Here's the drawing with two shaded views (mm, measured from the low corner). I have some questions. A direction names the side the tool comes from. Coordinates: 2 decimals unless noted, no trailing zeros. Loops run counter-clockwise (first coordinate to the right, second up) from the corner with the lowest first, then second, coordinate; pieces in that order, holes last.
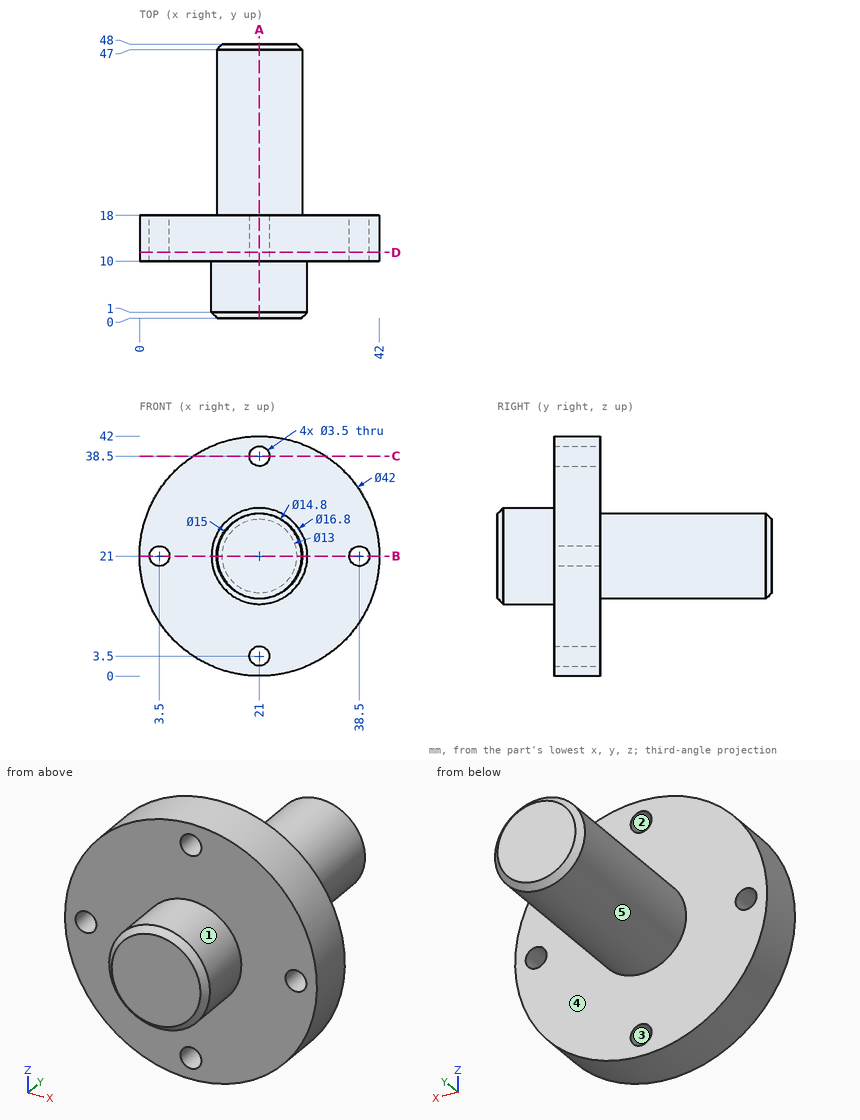
(1) I want a section at B-B on z = 21. Write out the boundary of the cut face in (x, y).
Check values:
outline: (0, 10) - (1.75, 10) - (1.75, 18) - (0, 18) - close; (5.25, 10) - (12.6, 10) - (12.6, 1) - (13.6, 0) - (28.4, 0) - (29.4, 1) - (29.4, 10) - (36.75, 10) - (36.75, 18) - (28.5, 18) - (28.5, 47) - (27.5, 48) - (14.5, 48) - (13.5, 47) - (13.5, 18) - (5.25, 18) - close; (40.25, 10) - (42, 10) - (42, 18) - (40.25, 18) - close
(2) I want a section at C-C on z = 38.5. Write out the boundary of the cut face in (x, y).
Check values:
outline: (9.39, 10) - (19.25, 10) - (19.25, 18) - (9.39, 18) - close; (22.75, 10) - (32.61, 10) - (32.61, 18) - (22.75, 18) - close
(3) I want a section at A-A on x = 21. Write out the boundary of the cut face in (y, z).
Check values:
outline: (0, 13.6) - (1, 12.6) - (10, 12.6) - (10, 5.25) - (18, 5.25) - (18, 13.5) - (47, 13.5) - (48, 14.5) - (48, 27.5) - (47, 28.5) - (18, 28.5) - (18, 36.75) - (10, 36.75) - (10, 29.4) - (1, 29.4) - (0, 28.4) - close; (10, 0) - (18, 0) - (18, 1.75) - (10, 1.75) - close; (10, 40.25) - (18, 40.25) - (18, 42) - (10, 42) - close
(4) If we mould it in two halves opening along X, with no side actions, what happens to the marked faces 3, 4 and 5? For each: released by +X, released by -X, zero draft, split by the parting line, or undercut.
Check values:
face 3: undercut
face 4: zero draft
face 5: split by the parting line
(5) If I drill on probe 1 along X at (y, z) = (12.5, 21); probe 2 along Y at (x, z) = (3.5, 11.5); probe 3 along Z at (x, y) = (39, 14.5), over which ranges is the centre line in solid material (lowest first)?
Check values:
probe 1: x = 0 to 1.75, 5.25 to 36.75, 40.25 to 42
probe 2: y = 10 to 18
probe 3: z = 10.18 to 19.32, 22.68 to 31.82
(6) Which directions (+Z, -Z, +X, -X, +Y, -Y) give clear straight access to the entire face, cutting with the end or side of a thin tool? Please do the marked faces 1 and 2.
Check values:
face 1: -Y
face 2: +Y, -Y
(7) I want a section at D-D on y = 11.5. Write out the boundary of the cut face in (x, z).
Check values:
outline: circle Ø42 at (21, 21); hole circle Ø3.5 at (3.5, 21); hole circle Ø3.5 at (21, 3.5); hole circle Ø3.5 at (21, 38.5); hole circle Ø3.5 at (38.5, 21)
(8) I'm going to push flat-ended pins straight in: pin 1 (8 mm diameter, centred on x = 9.5, z = 30.5, fed in from -Y); pin 2 (8 mm diameter, centred on x = 12, z = 27.5, fed in from +Y); pin 3 (8 mm diameter, centred on y = 7, z = 27.5, fed in from -X). Where does each tip first touch, or does it pass through?
Check values:
pin 1: stops at y = 10
pin 2: stops at y = 47.4
pin 3: stops at x = 0.36
